```python
from build123d import *

# Parameters (mm, degrees)
SKETCH_1_W             = 100
SKETCH_1_H             = 30
EXTRUDE_1_DEPTH        = 30
SKETCH_2_W             = 72
SKETCH_2_H             = 15
CUT_EXTRUDE_1_DEPTH    = 15.5
HOLE_WIZARD_M8_1_D     = 6.8
HOLE_WIZARD_M8_1_DEPTH = 10
HOLE_WIZARD_M8_1_TIP   = 2.042926105
HOLE_WIZARD_M5_1_D     = 4.2
CHAMFER_1_SIZE         = 5


with BuildPart() as part:
    # 草图1 → 凸台-拉伸1 (new body)
    with BuildSketch(Plane(origin=(0, 0, 0), x_dir=(0, 0, -1), z_dir=(1, 0, 0))):
        Rectangle(SKETCH_1_W, SKETCH_1_H)
    extrude(amount=EXTRUDE_1_DEPTH)

    # 草图2 → 切除-拉伸1 (cut)
    with BuildSketch(Plane(origin=(30, 0, 0), x_dir=(0, 0, -1), z_dir=(1, 0, 0))):
        with Locations((0, -7.5)):
            Rectangle(SKETCH_2_W, SKETCH_2_H)
    extrude(amount=-CUT_EXTRUDE_1_DEPTH, mode=Mode.SUBTRACT)

    # M8 螺纹孔1
    with Locations(Plane(origin=(0, 15, 0), x_dir=(1, 0, 0), z_dir=(0, 1, 0))):
        with Locations((15, 0), (15, 25), (15, -25)):
            Hole(HOLE_WIZARD_M8_1_D / 2, depth=HOLE_WIZARD_M8_1_DEPTH)
            with Locations((0, 0, -(HOLE_WIZARD_M8_1_DEPTH + HOLE_WIZARD_M8_1_TIP / 2))):  # 118° drill point
                Cone(0, HOLE_WIZARD_M8_1_D / 2, HOLE_WIZARD_M8_1_TIP, mode=Mode.SUBTRACT)

    # M5 螺纹孔1 (through all)
    with Locations(Plane(origin=(14.5, 0, 0), x_dir=(0, 0, -1), z_dir=(1, 0, 0))):
        with Locations((-20, -8), (0, -8), (20, -8)):
            Hole(HOLE_WIZARD_M5_1_D / 2)

    # 倒角1
    chamfer_1_edges = [part.edges().sort_by_distance(p)[0] for p in [
        (15, -15, -50),
        (15, -15, 50),
    ]]
    chamfer(chamfer_1_edges, length=CHAMFER_1_SIZE)


solid = part.part
```
Part model, mm, in its own coordinate system. A direction names the side the tool comes from. Round coordinates to 2 decimals unless told otherwise and drop trailing zeros. Loops run counter-clockwise (first coordinate to the right, second up) from the corner with the lowest first, then second, coordinate; pieces in that order, holes last. Notation, with made-up numbers: (-36.75, -17.5) -> (-0.75, -17.5) arc R23 cw to (-0.75, 21.5) -> close; hole circle Ø3 at (-22.5, 77). An arc over 180 degrees is marked (long way). Use a Markdown table: item, result.
1) Cut at B-B, the plane z = -20. List the corners of the cut face in (x, y).
The answers:
| item | result |
|---|---|
| outline | (0, -15) -> (14.5, -15) -> (14.5, -10.1) -> (0, -10.1) -> close; (0, -5.9) -> (14.5, -5.9) -> (14.5, 0) -> (30, 0) -> (30, 15) -> (0, 15) -> close |
2) Cut at A-A, the plane y = -8. List the corners of the cut face in (x, z), and give its area (3 significant figures).
The answers:
| item | result |
|---|---|
| outline | (0, -50) -> (30, -50) -> (30, -36) -> (14.5, -36) -> (14.5, -22.1) -> (0, -22.1) -> close; (0, -17.9) -> (14.5, -17.9) -> (14.5, -2.1) -> (0, -2.1) -> close; (0, 2.1) -> (14.5, 2.1) -> (14.5, 17.9) -> (0, 17.9) -> close; (0, 22.1) -> (14.5, 22.1) -> (14.5, 36) -> (30, 36) -> (30, 50) -> (0, 50) -> close |
| area | 1,700 mm2 |
3) Tool access for faces 4 (the flat face through (22, 0, 1)), 5 (the cylindrical face through (18.4, 9.9, -25.1)), 6 (the flat face through (11, 15, 1)): list every direction of +Z, -Z, +X, -X, +Y, -Y with a clear straight run to the whole face (end or side of a thin tool).
The answers:
| item | result |
|---|---|
| face 4 | +X, -Y |
| face 5 | +Y |
| face 6 | +Z, -Z, +X, -X, +Y |
4) Probe line 1 (Z direction, x = 15, y = 12.75); line 2 (X direction, y = 11.5, z = -25); line 3 (Z direction, x = 4, y = -9.25). List the from-to ranges inside material, lowest first. Write a range as [from, to].
The answers:
| item | result |
|---|---|
| line 1 | z = [-50, -28.4], [-21.6, -3.4], [3.4, 21.6], [28.4, 50] |
| line 2 | x = [0, 11.6], [18.4, 30] |
| line 3 | z = [-50, -21.69], [-18.31, -1.69], [1.69, 18.31], [21.69, 50] |
5) Drop flat-ended pins along their axis: pin 1 Ø3 at (x, z) = (19.5, -14) entering from -Y; pin 2 Ø6 at (y, z) = (-5.5, -21.5) entering from +X. Give the stop position or say it passes through.
The answers:
| item | result |
|---|---|
| pin 1 | stops at y = 0 |
| pin 2 | stops at x = 14.5 |
6) Cut at D-D, the plane y = 9.75. List the corners of the cut face in (x, z).
The answers:
| item | result |
|---|---|
| outline | (0, -50) -> (30, -50) -> (30, 50) -> (0, 50) -> close; hole circle Ø6.8 at (15, -25); hole circle Ø6.8 at (15, 0); hole circle Ø6.8 at (15, 25) |
7) Pull direction Y, two halves, no side cores. Call faces 1 (the cylindrical face through (7.148, -5.918, -0.273)), 2 (the flat face through (15, -13, 47)), 3 (the flat face through (22, -8, -36)): pulls with the +Y half, pulls with the -Y half, needs draft (parallel to the pull), parting line crosses it, or undercut.
The answers:
| item | result |
|---|---|
| face 1 | undercut |
| face 2 | pulls with the -Y half |
| face 3 | needs draft |
8) Cut at C-C, the plane x = 7.5. List the corners of the cut face in (y, z), and give its area (3 significant figures).
The answers:
| item | result |
|---|---|
| outline | (-15, -45) -> (-10, -50) -> (15, -50) -> (15, 50) -> (-10, 50) -> (-15, 45) -> close; hole circle Ø4.2 at (-8, -20); hole circle Ø4.2 at (-8, 0); hole circle Ø4.2 at (-8, 20) |
| area | 2,930 mm2 |
